For this review, take the finished solid that the model builds, in its own axes (mm). A direction names the side the tool comes from. Give positions to 0.01 mm unless a question says otherwise; leave off trailing zeros. Write each loop counter-clockwise with the first axis right and the second up, starting at its lowest first coordinate (ties: lowest second). Pieces come first, ordered by that corner, then holes. Notation, with made-up numbers: M -31.75,80.5 L -4.75,80.5 A33 ccw -4.75,110.5 Z; hole C -20.5,-40 d10. An arc over 180 degrees is marked long. Answer as a JSON object with one key per item and string values. Group by question number.
```python
from build123d import *

# Parameters (mm, degrees)
BOSS_EXTRUDE1_DEPTH = 11.25
SKETCH2_R           = 1.317449136
SKETCH2_R_2         = 1.488469479
CUT_EXTRUDE1_DEPTH  = 2


with BuildPart() as part:
    # Sketch1 → Boss-Extrude1 (new, symmetric)
    with BuildSketch(Plane(origin=(0, 0, 0), x_dir=(0, 0, -1), z_dir=(1, 0, 0))):
        Polygon((-8.258522727, 5.046875), (8.741477273, 5.046875), (8.741477273, -1.453125), (3.741477273, -1.453125), (3.741477273, 2.046875), (-3.258522727, 2.046875), (-3.258522727, -1.453125), (-8.258522727, -1.453125), align=None)
    extrude(amount=BOSS_EXTRUDE1_DEPTH, both=True)

    # Sketch2 → Cut-Extrude1 (cut)
    with BuildSketch(Plane(origin=(0, 5.046875, 0), x_dir=(1, 0, 0), z_dir=(0, 1, 0))):
        with Locations(Location((4, -5.758522727, 0), (0, 0, 270))):
            Circle(SKETCH2_R)
        with Locations(Location((-4, 6.241477273, 0), (0, 0, 270))):
            Circle(SKETCH2_R_2)
        with Locations(Location((4, 6.241477273, 0), (0, 0, 90))):
            Circle(SKETCH2_R_2)
        with Locations(Location((-4, -5.758522727, 0), (0, 0, 90))):
            Circle(SKETCH2_R)
    extrude(amount=-CUT_EXTRUDE1_DEPTH, mode=Mode.SUBTRACT)


solid = part.part
```
Item 1: Consider section A-A (y = 1.75). Give the boundary of the cut face in (x, z), plus the area to 3 significant figures.
Item 2: Consider section B-B (y = 4.5). Give the boundary of the cut face in (x, z).
Item 3: Machinability: for faces 4 (the cylindrical face through (2.994, 4.061, -5.144)), 5 (the flat face through (0, 0, 3.259)), 6 (the flat face through (0, 2, -8.741)), which of the approach directions +Z, -Z, +X, -X, +Y, -Y give a long, thin tool a straight path to every point of the face, cutting with its end or side? Answer none if there is none.
Item 4: Consider section D-D (x = -4). Give the boundary of the cut face in (y, z).
Item 5: Draft analysis for pull direction X (two halves, no side actions). For faces 1 (the flat face through (0, 2.047, 0)), 2 (the flat face through (-4, 3.047, -6)), 3 (the flat face through (-11.25, 3, 0)), state which applies: released by +X, released by -X, zero draft, split by the parting line, or undercut.
Item 6: To check wall thickness, follow probe 1 along Z at (x, y) = (0, 0.5); probe 2 along X at (y, z) = (4, -5.75); probe 3 along Y at (x, z) = (-1.75, 1). State the ranges of each line that lie inside material, in increasing order.
Item 7: Insertion check: P1, Ø1.6, axis at x = -4, z = 5.76, coming from the +Y side. The pin has a flat end and moves straight along its axis. Give the tip position at first contact, or say it passes through.
Item 8: Consider section C-C (x = 5.75). Give the boundary of the cut face in (y, z).
Result set:
{
 "1": {"outline": "M -11.25,-8.74 L 11.25,-8.74 L 11.25,-3.74 L -11.25,-3.74 Z; M -11.25,3.26 L 11.25,3.26 L 11.25,8.26 L -11.25,8.26 Z", "area": "225 mm^2"},
 "2": {"outline": "M -11.25,-8.74 L 11.25,-8.74 L 11.25,8.26 L -11.25,8.26 Z; hole C -4,-6.24 d2.98; hole C -4,5.76 d2.63; hole C 4,-6.24 d2.98; hole C 4,5.76 d2.63"},
 "3": {"face 4": "+Y", "face 5": "+X, -X, -Y", "face 6": "-Z, +X, -X, +Y, -Y"},
 "4": {"outline": "M -1.45,-8.74 L 5.05,-8.74 L 5.05,-7.73 L 3.05,-7.73 L 3.05,-4.75 L 5.05,-4.75 L 5.05,4.44 L 3.05,4.44 L 3.05,7.08 L 5.05,7.08 L 5.05,8.26 L -1.45,8.26 L -1.45,3.26 L 2.05,3.26 L 2.05,-3.74 L -1.45,-3.74 Z"},
 "5": {"face 1": "zero draft", "face 2": "undercut", "face 3": "released by -X"},
 "6": {"probe 1": "z = -8.74 to -3.74, 3.26 to 8.26", "probe 2": "x = -11.25 to -5.4, -2.6 to 2.6, 5.4 to 11.25", "probe 3": "y = 2.05 to 5.05"},
 "7": {"P1": "stops at y = 3.05"},
 "8": {"outline": "M -1.45,-8.74 L 5.05,-8.74 L 5.05,8.26 L -1.45,8.26 L -1.45,3.26 L 2.05,3.26 L 2.05,-3.74 L -1.45,-3.74 Z"}
}
